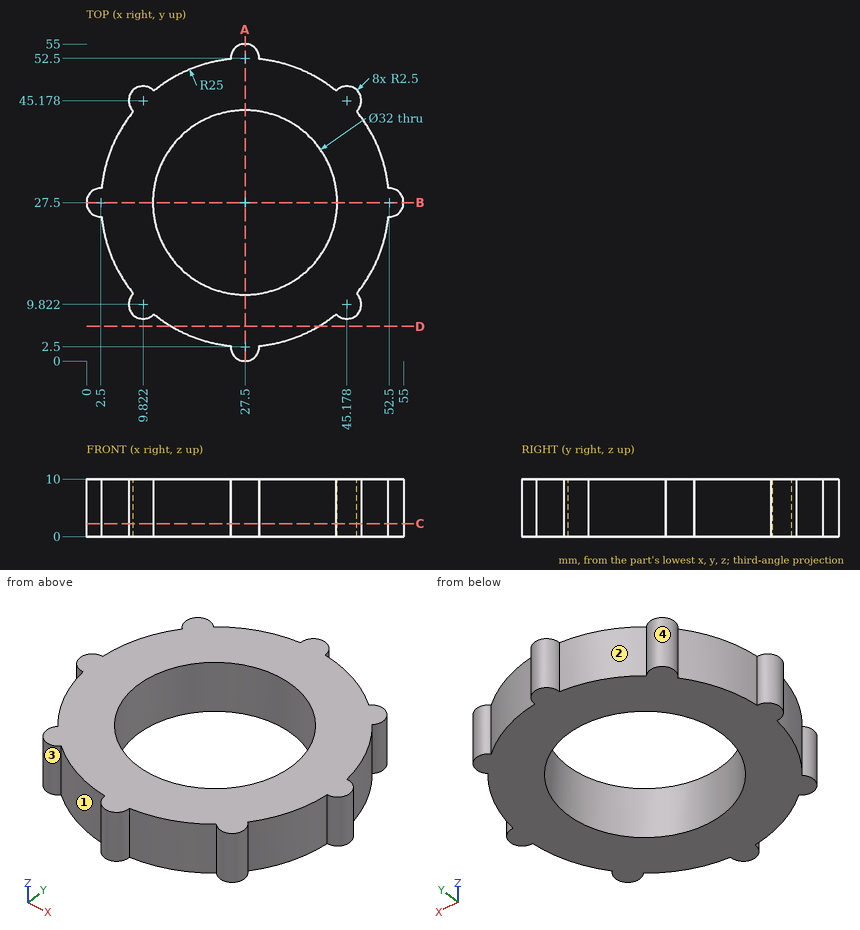
Print and shaded views of the part. All mm, measured from the part's lowest x, y and z. Round coordinates to 2 decimals unless told otherwise and drop trailing zeros. Write each loop counter-clockwise with the first axis right and the second up, starting at its lowest first coordinate (ties: lowest second). Pieces come first, ordered by that corner, then holes. Notation, with made-up numbers: M 28.25,66 L 33.25,66 A5 cw 33.25,73 Z; hole C 37,-34 d8. An arc over 180 degrees is marked long. Use a Markdown table: item, result. Add a question column.
1. Flat gauge pins, fed straight in: P1, Ø3, axis at x = 42, z = 1.5, coming from the +Y side (1 decimal); P2, Ø2, axis at x = 8.5, z = 2.5, coming from the +Y side; P3, Ø3, axis at x = 19.5, z = 3.5, coming from the -Y side. Where does each tip first touch, or does it go through?
2. Slice it at A-A on x = 27.5. Give the cut face in (y, z), then the cut area to 3 significant figures.
3. Slice it at C-C on z = 2.25. Give the cut face in (x, y) (1 decimal), then the cut area to 3 significant figures.
4. Slice it at D-D on y = 6. Give the cut face in (x, z), then the cut area to 3 significant figures.
5. Pull direction Y, two halves, no side cores. Call the marked faces 1, 2, 3 and 4: released by +Y, released by -Y, zero draft, split by the parting line, or undercut.
6. Drill centre lines: probe 1 along Y at (x, z) = (27.5, 7.75); probe 2 along Y at (x, z) = (8, 8.25) (1 decimal); probe 3 along X at (y, z) = (16.5, 0.5). Where is each one in solid material? Low to high.
Reply:
| question | item | result |
|---|---|---|
| 1 | P1 | stops at y = 48.9 |
| 1 | P2 | stops at y = 47.66 |
| 1 | P3 | stops at y = 3.36 |
| 2 | outline | M 0,0 L 11.5,0 L 11.5,10 L 0,10 Z; M 43.5,0 L 55,0 L 55,10 L 43.5,10 Z |
| 2 | area | 230 mm^2 |
| 3 | outline | M 2.6,25 A25 ccw 8.1,11.7 A2.5 ccw long 11.7,8.1 A25 ccw 25,2.6 A2.5 ccw long 30,2.6 A25 ccw 43.3,8.1 A2.5 ccw long 46.9,11.7 A25 ccw 52.4,25 A2.5 ccw long 52.4,30 A25 ccw 46.9,43.3 A2.5 ccw long 43.3,46.9 A25 ccw 30,52.4 A2.5 ccw long 25,52.4 A25 ccw 11.7,46.9 A2.5 ccw long 8.1,43.3 A25 ccw 2.6,30 A2.5 ccw long Z; hole C 27.5,27.5 d32 |
| 3 | area | 1,240 mm^2 |
| 4 | outline | M 14.74,0 L 40.26,0 L 40.26,10 L 14.74,10 Z |
| 4 | area | 255 mm^2 |
| 5 | face 1 | released by -Y |
| 5 | face 2 | released by +Y |
| 5 | face 3 | undercut |
| 5 | face 4 | undercut |
| 6 | probe 1 | y = 0 to 11.5, 43.5 to 55 |
| 6 | probe 2 | y = 8.1 to 11.5, 11.9 to 43.1, 43.5 to 46.9 |
| 6 | probe 3 | x = 5.05 to 15.88, 39.12 to 49.95 |
